from build123d import *

# Parameters (mm, degrees)
SKETCH_1_R      = 3
EXTRUDE_1_DEPTH = 14
SKETCH_2_R      = 6
EXTRUDE_2_DEPTH = 4
CHAMFER_1_SIZE  = 1
EXTRUDE_START   = 4
SKETCH_3_R      = 6
EXTRUDE_3_DEPTH = 4
CHAMFER_2_SIZE  = 1


with BuildPart() as part:
    # 草图1 → 凸台-拉伸1 (new body)
    with BuildSketch(Plane.XY):
        Circle(SKETCH_1_R)
    extrude(amount=EXTRUDE_1_DEPTH)

    # 草图2 → 凸台-拉伸2 (add)
    with BuildSketch(Plane.XY.offset(14)):
        Circle(SKETCH_2_R)
    extrude(amount=EXTRUDE_2_DEPTH)

    # 倒角1
    chamfer_1_edges = [part.edges().sort_by_distance(p)[0] for p in [
        (-6, 0, 18),
    ]]
    chamfer(chamfer_1_edges, length=CHAMFER_1_SIZE)

    # 草图3 → 凸台-拉伸3 (add)
    with BuildSketch(Plane(origin=(0, 0, 0), x_dir=(-1, 0, 0), z_dir=(0, 0, -1)).offset(EXTRUDE_START)):
        with Locations(Location((0, 0, 0), (0, 0, 180))):
            Circle(SKETCH_3_R)
    extrude(amount=-EXTRUDE_3_DEPTH)

    # 倒角2
    chamfer_2_edges = [part.edges().sort_by_distance(p)[0] for p in [
        (-6, 0, -4),
    ]]
    chamfer(chamfer_2_edges, length=CHAMFER_2_SIZE)


solid = part.part
Build history of the part. All positions in model axes, mm. A direction names the side the tool comes from. Coordinates: 2 decimals unless noted, no trailing zeros. Order: outer loops, then holes, each group sorted by start corner. A loop starts at its lowest first (then second) coordinate and runs counter-clockwise, first axis right, second up. Notation, with made-up numbers: M 31.25,-24 L 66.25,-24 A31 ccw 66.25,15 Z; hole C 5,-18 d2. An arc over 180 degrees is marked long. One line per question, with ' | ' between items. Start each with the question number.
Q1. Flat gauge pins, fed straight in: pin 1 Ø2 at (y, z) = (-3, -1) entering from -X; pin 2 Ø5 at (x, z) = (-4, 1) entering from +Y; pin 3 Ø1 at (x, z) = (-1, 1) entering from +Y. Where does each tip first touch, or does it go through?
Q2. Saw through at A-A (x = 0). List the corners of the cut face in (y, z).
Q3. Saw through at C-C (z = 11.25). List the corners of the cut face in (x, y).
Q4. Two-plate mould, pull along Z, no slides. Class faces 3 (the face through (0, 0, -4)), 4 (the face through (5.723, -1.802, -1.521)), 5 (the face through (-3, 0, 7)): +Z half, -Z half, draft (parallel to the pull), parting line (faces both ways), or undercut.
Q5. Probe L1, parallel to Z at x = -1, y = -4; L2, parallel to Z at x = -4.75, y = -2.5; L3, parallel to Y at x = -0.25, z = 5.75. List the from-to ranges inside material, lowest first. Write a range as from..to.
Q6. 3-axis set-ups, long thin cutter, end or side, ignore diameter. For faces 1 (the face through (-6, 0, 15)), 2 (the face through (-3, -1, 14)): which of +Z, -Z, +X, -X, +Y, -Y reach the whole face in a straight line?
Check values:
1) pin 1: stops at x = -5.66 | pin 2: stops at y = 5.75 | pin 3: stops at y = 2.96
2) outline: M -6,-3 L -5,-4 L 5,-4 L 6,-3 L 6,0 L 3,0 L 3,14 L 6,14 L 6,17 L 5,18 L -5,18 L -6,17 L -6,14 L -3,14 L -3,0 L -6,0 Z
3) outline: C 0,0 d6
4) face 3: -Z half | face 4: draft | face 5: undercut
5) L1: z = -4..0, 14..18 | L2: z = -3.63..0, 14..17.63 | L3: y = -2.99..2.99
6) face 1: +Z, -Z | face 2: none
